Verification items for this drawing (mm, ordinates from the low corner). A direction names the side the tool comes from. Coordinates: 2 decimals unless noted, no trailing zeros. Write each loop counter-clockwise with the first axis right and the second up, starting at its lowest first coordinate (ties: lowest second). Pieces come first, ordered by that corner, then holes. Notation, with made-up numbers: M -14.5,12 L 20.5,12 A22 ccw 20.5,47 Z; hole C -27,55.5 d8. An arc over 180 degrees is marked long. Answer as CSV lines item,"result". Start each with the question number.
1) Section check C-C (y = 3.3). Record the cut outline in (x, z).
2) Material ranges on L1, parallel to X at y = 2.6, z = 12; L2, parallel to Z at x = 11.75, y = 4.7 (1 decimal); L3, parallel to Y at x = 14, z = 21.75 (1 decimal), recorded low to high. Write a range as [from, to].
3) Go/stop test with flat-tipped pins: pin 1 Ø9.5 at (x, z) = (12, 12) entering from -Y; pin 2 Ø1 at (y, z) = (2.5, 4) entering from -X; pin 3 Ø3 at (y, z) = (1.5, 7) entering from -X; pin 4 Ø2 at (y, z) = (2, 18.5) entering from +X (1 decimal). Record where each tip stops, or that it passes through.
4) Draft check along X on the marked faces 1, 2 and 3. Enter one of: +X half, -X half, draft (parallel to the pull), parting line (faces both ways), or undercut.
5) Access from +Z, -Z, +X, -X, +Y, -Y to the whole of each face (thin tool, end or side, straight path). Record for the marked faces 4, 5 and 6.
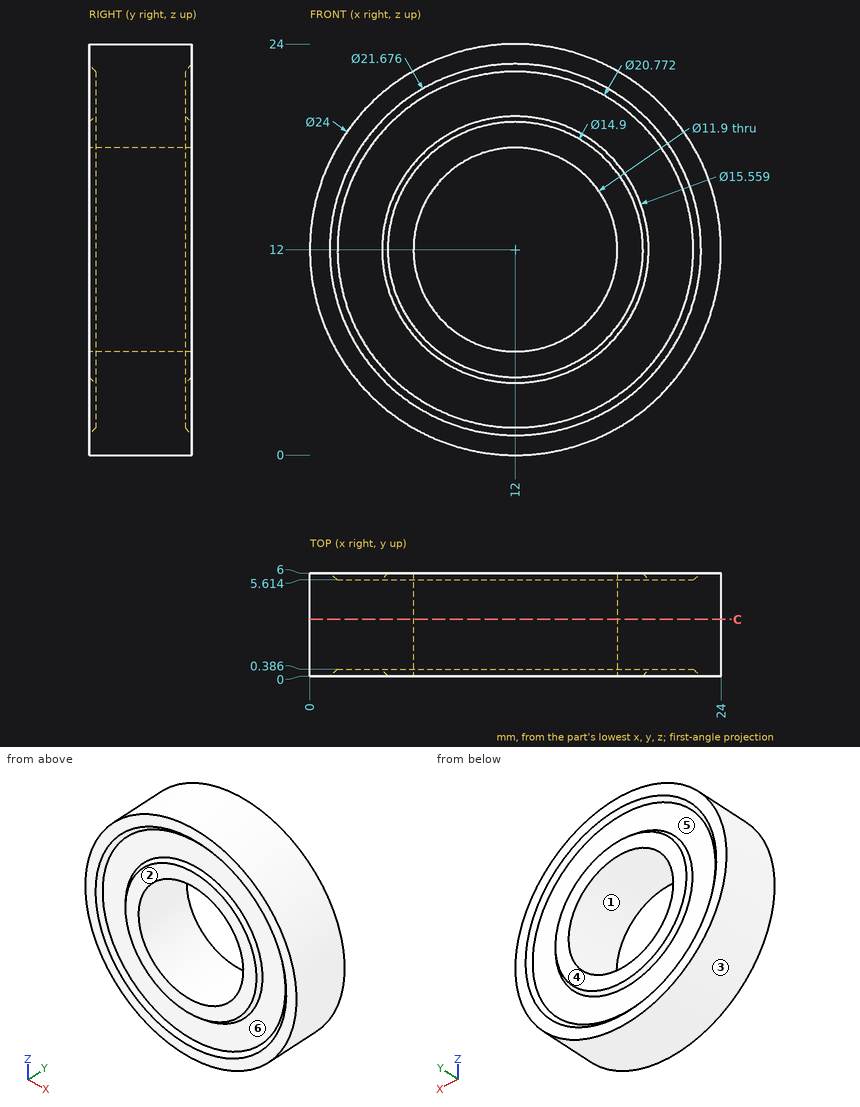
Results found:
1,outline,"C 12,12 d24; hole C 12,12 d11.9"
2,L1,"x = [0, 6.05], [17.95, 24]"
2,L2,"z = [0, 6.1], [17.9, 24]"
2,L3,"y = [0.4, 5.6]"
3,pin 1,"passes through"
3,pin 2,"stops at x = 2.63"
3,pin 3,"stops at x = 0.52"
3,pin 4,"stops at x = 22.7"
4,face 1,"undercut"
4,face 2,"draft"
4,face 3,"parting line"
5,face 4,"+Z, -Z, +X, -X, +Y"
5,face 5,"+Y"
5,face 6,"-Y"
